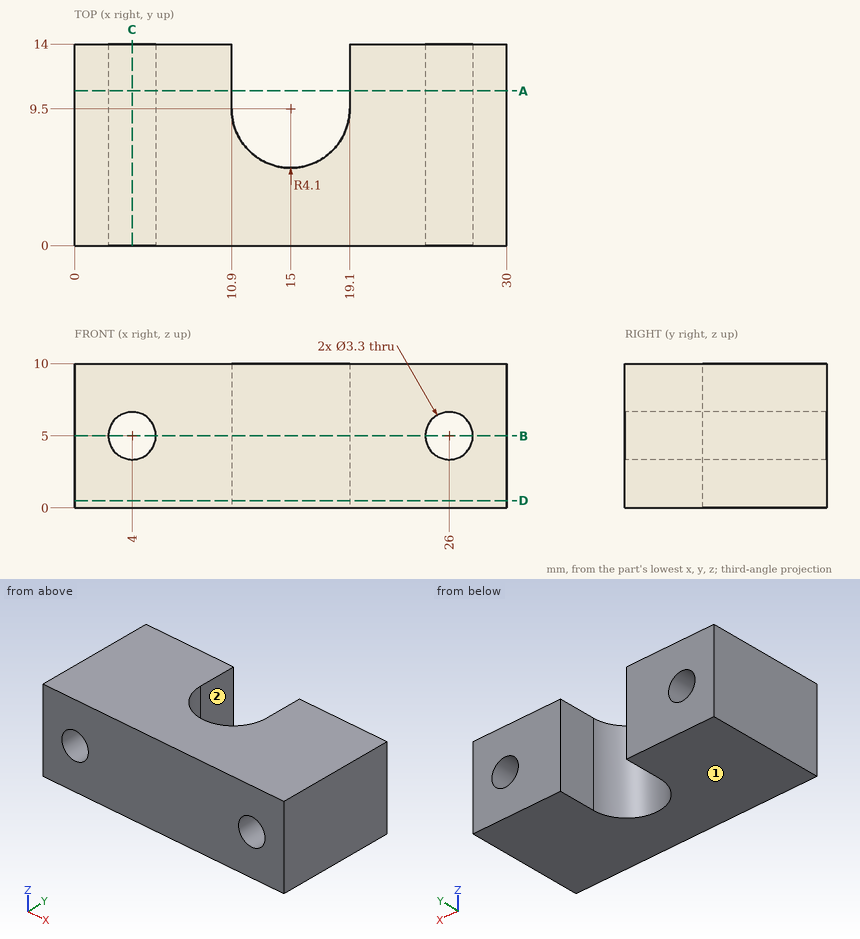
Part print with two shaded views. Sizes in mm from the minimum x, y, z corner. A direction names the side the tool comes from. Round coordinates to 2 decimals unless told otherwise and drop trailing zeros. Order: outer loops, then holes, each group sorted by start corner. A loop starts at its lowest first (then second) coordinate and runs counter-clockwise, first axis right, second up. Notation, with made-up numbers: M 27,20 L 40,20 A33 ccw 40,49 Z; hole C 51.5,54 d4. An arc over 180 degrees is marked long. Put each result on its own line as item: value. Start each with the question number.
1. Tool access for the marked faces 1 and 2: list every direction of +Z, -Z, +X, -X, +Y, -Y with a clear straight run to the whole face (end or side of a thin tool).
2. Slice it at B-B on z = 5. List the corners of the cut face in (x, y), then the cut area to 3 significant figures.
3. Slice it at C-C on x = 4. List the corners of the cut face in (y, z), then the cut area to 3 significant figures.
4. Drill centre lines: probe 1 along X at (y, z) = (10.25, 5); probe 2 along X at (y, z) = (5.25, 5); probe 3 along X at (y, z) = (7.5, 5). Where is each one in solid material? Low to high. Write a range as [from, to].
5. Slice it at A-A on y = 10.75. List the corners of the cut face in (x, z).
6. Slice it at D-D on z = 0.5. List the corners of the cut face in (x, y), then the cut area to 3 significant figures.
Findings:
1. face 1: -Z, +X, -X, +Y, -Y
1. face 2: +Z, -Z, +Y
2. outline: M 0,0 L 2.35,0 L 2.35,14 L 0,14 Z; M 5.65,0 L 24.35,0 L 24.35,14 L 19.1,14 L 19.1,9.5 A4.1 cw 10.9,9.5 L 10.9,14 L 5.65,14 Z; M 27.65,0 L 30,0 L 30,14 L 27.65,14 Z
2. area: 264 mm2
3. outline: M 0,0 L 14,0 L 14,3.35 L 0,3.35 Z; M 0,6.65 L 14,6.65 L 14,10 L 0,10 Z
3. area: 93.8 mm2
4. probe 1: [0, 2.35], [5.65, 10.9], [19.1, 24.35], [27.65, 30]
4. probe 2: [0, 2.35], [5.65, 24.35], [27.65, 30]
4. probe 3: [0, 2.35], [5.65, 11.42], [18.58, 24.35], [27.65, 30]
5. outline: M 0,0 L 10.9,0 L 10.9,10 L 0,10 Z; M 19.1,0 L 30,0 L 30,10 L 19.1,10 Z; hole C 4,5 d3.3; hole C 26,5 d3.3
6. outline: M 0,0 L 30,0 L 30,14 L 19.1,14 L 19.1,9.5 A4.1 cw 10.9,9.5 L 10.9,14 L 0,14 Z
6. area: 357 mm2
